The model under review builds one solid part; all positions refer to its coordinate system, in mm. Round coordinates to 2 decimals unless told otherwise and drop trailing zeros. Order: outer loops, then holes, each group sorted by start corner. A loop starts at its lowest first (then second) coordinate and runs counter-clockwise, first axis right, second up.
from build123d import *

# Parameters (mm, degrees)
SKETCH1_W           = 350
SKETCH1_H           = 60
SKETCH1_R           = 3.25
BOSS_EXTRUDE1_DEPTH = 10
M10_TAPPED_HOLE1_D  = 8.5


with BuildPart() as part:
    # Sketch1 → Boss-Extrude1 (new body)
    with BuildSketch(Plane.XY):
        with Locations((0, 30)):
            Rectangle(SKETCH1_W, SKETCH1_H)
        with Locations((-145, 47.5)):
            Circle(SKETCH1_R, mode=Mode.SUBTRACT)
        with Locations((-110, 47.5)):
            Circle(SKETCH1_R, mode=Mode.SUBTRACT)
        with Locations(Location((-110, 12.5, 0), (0, 0, 180))):
            Circle(SKETCH1_R, mode=Mode.SUBTRACT)
        with Locations(Location((-145, 12.5, 0), (0, 0, 180))):
            Circle(SKETCH1_R, mode=Mode.SUBTRACT)
        with Locations((110, 12.5)):
            Circle(SKETCH1_R, mode=Mode.SUBTRACT)
        with Locations((145, 12.5)):
            Circle(SKETCH1_R, mode=Mode.SUBTRACT)
        with Locations(Location((110, 47.5, 0), (0, 0, 180))):
            Circle(SKETCH1_R, mode=Mode.SUBTRACT)
        with Locations(Location((145, 47.5, 0), (0, 0, 180))):
            Circle(SKETCH1_R, mode=Mode.SUBTRACT)
    extrude(amount=BOSS_EXTRUDE1_DEPTH)

    # M10 Tapped Hole1 (through all)
    with Locations(Plane.XY.offset(10)):
        with Locations((-35, 12), (35, 12)):
            Hole(M10_TAPPED_HOLE1_D / 2)


solid = part.part
(1) Clearance check with a flat-ended pin moving along its axis: P1, Ø4, axis at x = 110, y = 47.5, coming from the +Z side. State where the tip first meets the part, or that it passes through.
(2) To check wall thickness, follow L1, parallel to Y at x = -110, z = 2.75; L2, parallel to X at y = 50, z = 1.25; L3, parallel to X at y = 49.5, z = 3.5. State the ranges of each line that lie inside material, in increasing order.
(3) The part is to be moulded in two halves that separate along Y. For faces 1 (the flat face through (-2, 0, 5)), 2 (the flat face through (-2, 60, 5)), 3 (the flat face through (175, 30, 5)), 4 (the cylindrical face through (39.246, 12.187, 4.93)), say which applies: pulls with the +Y half, pulls with the -Y half, needs draft (parallel to the pull), parting line crosses it, or undercut.
(4) We need section B-B (x = -110). Give the boundary of the cut face in (y, z), and give its area (3 significant figures).
(5) We need section C-C (x = 35). Give the boundary of the cut face in (y, z), and give its area (3 significant figures).
(6) We need section A-A (z = 2.5). Count the separate pieces of the cut face and the enclosed holes in it, and give its area (3 significant figures).
Verdict:
1. P1: passes through
2. L1: y = 0 to 9.25, 15.75 to 44.25, 50.75 to 60
2. L2: x = -175 to -147.08, -142.92 to -112.08, -107.92 to 107.92, 112.08 to 142.92, 147.08 to 175
2. L3: x = -175 to -147.56, -142.44 to -112.56, -107.44 to 107.44, 112.56 to 142.44, 147.56 to 175
3. face 1: pulls with the -Y half
3. face 2: pulls with the +Y half
3. face 3: needs draft
3. face 4: undercut
4. outline: (0, 0) - (9.25, 0) - (9.25, 10) - (0, 10) - close; (15.75, 0) - (44.25, 0) - (44.25, 10) - (15.75, 10) - close; (50.75, 0) - (60, 0) - (60, 10) - (50.75, 10) - close
4. area: 470 mm2
5. outline: (0, 0) - (7.75, 0) - (7.75, 10) - (0, 10) - close; (16.25, 0) - (60, 0) - (60, 10) - (16.25, 10) - close
5. area: 515 mm2
6. separate pieces: 1
6. enclosed holes: 10
6. area: 20,600 mm2
